CAD build for the part. Positions are in the model's coordinates, mm. Face numbers are marked on the shaded views. A direction names the side the tool comes from. Coordinates: 2 decimals unless noted, no trailing zeros. Write each loop counter-clockwise with the first axis right and the second up, starting at its lowest first coordinate (ties: lowest second). Pieces come first, ordered by that corner, then holes. Notation, with made-up numbers: (41, 80.25) - (50, 80.25) arc R20 ccw to (50, 90.25) - close; hole circle Ø2 at (44.25, -16). An arc over 180 degrees is marked (long way). One line per question, with ' | ' between items. Start each with the question number.
1. Flat gauge pins, fed straight in: P1, Ø2, axis at x = 0.5, z = 0.5, coming from the +Y side; P2, Ø1, axis at y = -9.5, z = 1, coming from the -X side; P3, Ø1.8, axis at y = -19.5, z = 2, coming from the +X side. Where does each tip first touch, or does it go through?
2. Probe line 1 (X direction, y = 0, z = 0.55); line 2 (Y direction, x = -1.5, z = 3); line 3 (Y direction, x = -2, z = 1.7). List the from-to ranges inside material, lowest first.
3. Band-saw the part on A-A, the plane x = 0. Write the cut outline in (y, z).
4. Two-plate mould, pull along X, no slides. Class the marked faces 1, 2 and 3: +X half, -X half, draft (parallel to the pull), parting line (faces both ways), or undercut.
5. Band-saw the part on D-D, the plane y = 7.5. Give the number of separate pieces and of enclosed holes in the cut face, then the cut area to 3 significant figures.
6. Which spindle directions (+Z, -Z, +X, -X, +Y, -Y) get a long thin tool onto all of the face, cutting with end or side? Do the marked faces 4, 5 and 6. Say none if no direction does.
7. Band-saw the part on B-B, the plane y = 0. Write the cut outline in (x, z).
8. Band-saw the part on C-C, the plane z = 1.7. Write the cut outline in (x, y), then the cut area to 3 significant figures.
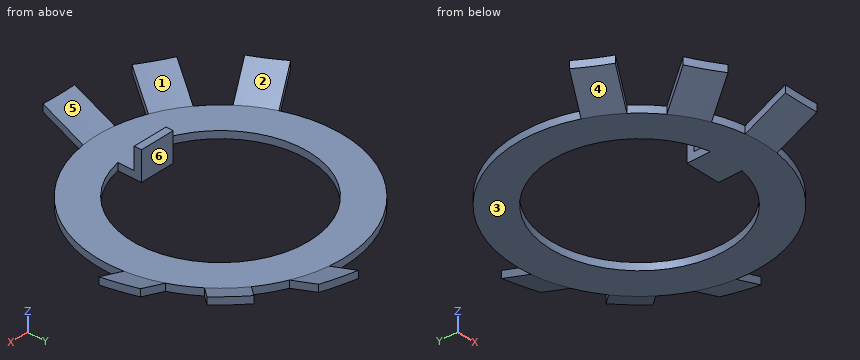
from build123d import *

# Parameters (mm, degrees)
CUT_EXTRUDE2_START  = -3e-06
SKETCH3_OUTSIDE_W   = 59.748
SKETCH3_OUTSIDE_H   = 59.748
CUT_EXTRUDE2_DEPTH  = 3.564697
SKETCH4_W           = 4.8
SKETCH4_H           = 1
BOSS_EXTRUDE1_DEPTH = 4


with BuildPart() as part:
    # Sketch2 → Boss-Revolve (revolve)
    with BuildSketch(Plane(origin=(0, 0, 0), x_dir=(0, 0, -1), z_dir=(1, 0, 0))):
        Polygon((-2.56469212, 22.5), (0, 17), (0, 0), (-1, 0), (-1, 17), (-3.56469212, 22.5), align=None)
    revolve(axis=Axis((0, 0, 0), (0, 0, 1)))

    # Sketch3 outside → Cut-Extrude2 (cut)
    # profile 1 of 2: a face of its own
    with BuildSketch(Plane.XY.offset(CUT_EXTRUDE2_START)):
        Rectangle(SKETCH3_OUTSIDE_W, SKETCH3_OUTSIDE_H)
        with BuildLine():
            Line((-2.4, -16.829735589), (-2.4, -22.371633825))
            Line((-2.4, -22.371633825), (2.4, -22.371633825))
            Line((2.4, -22.371633825), (2.4, -16.829735589))
            ThreePointArc((2.4, -16.829735589), (13.487006785, -10.348944293), (16.877441963, 2.037634111))
            Line((16.877441963, 2.037634111), (22.230504596, 3.471982921))
            Line((22.230504596, 3.471982921), (20.98817318, 8.108426887))
            Line((20.98817318, 8.108426887), (15.635110547, 6.674078078))
            ThreePointArc((15.635110547, 6.674078078), (14.722431864, 8.5), (13.597476435, 10.203363886))
            Line((13.597476435, 10.203363886), (17.516190259, 14.122077709))
            Line((17.516190259, 14.122077709), (14.122077709, 17.516190259))
            Line((14.122077709, 17.516190259), (10.203363886, 13.597476435))
            ThreePointArc((10.203363886, 13.597476435), (8.5, 14.722431864), (6.674078078, 15.635110547))
            Line((6.674078078, 15.635110547), (8.108426887, 20.98817318))
            Line((8.108426887, 20.98817318), (3.471982921, 22.230504596))
            Line((3.471982921, 22.230504596), (2.037634111, 16.877441963))
            ThreePointArc((2.037634111, 16.877441963), (-13.487006785, 10.348944293), (-15.774978559, -6.336406825))
            Line((-15.774978559, -6.336406825), (-20.574403217, -9.107355943))
            Line((-20.574403217, -9.107355943), (-18.174403217, -13.264277882))
            Line((-18.174403217, -13.264277882), (-13.374978559, -10.493328764))
            ThreePointArc((-13.374978559, -10.493328764), (-12.02081528, -12.02081528), (-10.493328764, -13.374978559))
            Line((-10.493328764, -13.374978559), (-13.264277882, -18.174403217))
            Line((-13.264277882, -18.174403217), (-9.107355943, -20.574403217))
            Line((-9.107355943, -20.574403217), (-6.336406825, -15.774978559))
            ThreePointArc((-6.336406825, -15.774978559), (-4.399923767, -16.420739047), (-2.4, -16.829735589))
        make_face(mode=Mode.SUBTRACT)
    # profile 2 of 2: a face of its own
    with BuildSketch(Plane.XY.offset(CUT_EXTRUDE2_START)):
        with BuildLine():
            Line((2.4, -12.012597554), (2.4, -8.75))
            Line((2.4, -8.75), (-2.4, -8.75))
            Line((-2.4, -8.75), (-2.4, -12.012597554))
            ThreePointArc((-2.4, -12.012597554), (0, 12.25), (2.4, -12.012597554))
        make_face()
    extrude(amount=CUT_EXTRUDE2_DEPTH, mode=Mode.SUBTRACT)

    # Sketch4 → Boss-Extrude1 (add)
    with BuildSketch(Plane.XY):
        with Locations((0, -9.25)):
            Rectangle(SKETCH4_W, SKETCH4_H)
    extrude(amount=BOSS_EXTRUDE1_DEPTH)


solid = part.part
Filled in:
1) P1: stops at y = 17 | P2: stops at x = -17.87 | P3: stops at x = 2.4
2) line 1: x = -17 to -12.25, 12.25 to 17 | line 2: y = -22.37 to -21.24, -9.75 to -8.75 | line 3: y = -20.55 to -18.39, -9.75 to -8.75
3) outline: (-22.37, 2.5) - (-17, 0) - (-8.75, 0) - (-8.75, 4) - (-9.75, 4) - (-9.75, 1) - (-17, 1) - (-22.37, 3.5) - close; (12.25, 0) - (17, 0) - (17, 1) - (12.25, 1) - close
4) face 1: +X half | face 2: undercut | face 3: draft
5) separate pieces: 3 | enclosed holes: 0 | area: 13.6 mm²
6) face 4: -Z, -X, -Y | face 5: +Z | face 6: +Z, -Z
7) outline: (-17, 0) - (-12.25, 0) - (-12.25, 1) - (-17, 1) - close; (12.25, 0) - (17, 0) - (17, 1) - (12.25, 1) - close
8) outline: (-18.96, -8.17) arc R20.65 ccw to (-16.56, -12.33) - (-14.69, -11.25) arc R18.5 cw to (-17.09, -7.09) - close; (-12.33, -16.56) arc R20.65 ccw to (-8.17, -18.96) - (-7.09, -17.09) arc R18.5 cw to (-11.25, -14.69) - close; (-2.4, -20.51) arc R20.65 ccw to (2.4, -20.51) - (2.4, -18.34) arc R18.5 cw to (-2.4, -18.34) - close; (-2.4, -9.75) - (2.4, -9.75) - (2.4, -8.75) - (-2.4, -8.75) - close; (2.43, 18.34) arc R18.5 cw to (7.07, 17.1) - (7.63, 19.19) arc R20.65 ccw to (2.99, 20.43) - close; (11.27, 14.67) arc R18.5 cw to (14.67, 11.27) - (16.2, 12.8) arc R20.65 ccw to (12.8, 16.2) - close; (17.1, 7.07) arc R18.5 cw to (18.34, 2.43) - (20.43, 2.99) arc R20.65 ccw to (19.19, 7.63) - close | area: 66.7 mm²
